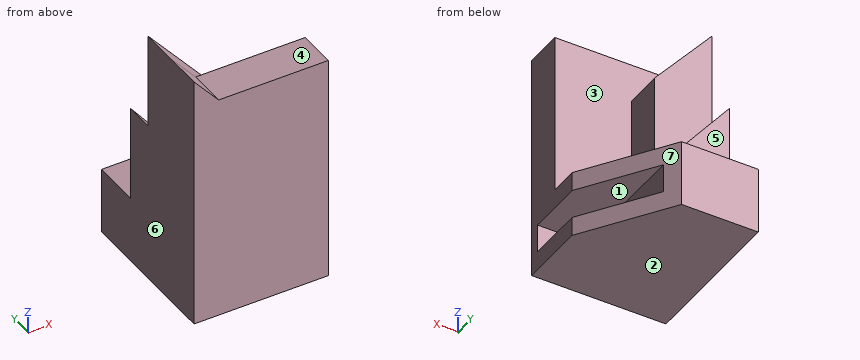
from build123d import *

# Parameters (mm, degrees)
BASE_PLATE_SKETCH_W   = 70
BASE_PLATE_SKETCH_H   = 135
BASE_PLATE_DEPTH      = 20
TOWER_DEPTH           = 35
TOWER_WINDOW_SKETCH_W = 25
TOWER_WINDOW_SKETCH_H = 15
TOWER_WINDOW_DEPTH    = 75
UPPER_STEP_DEPTH      = 35
LOWER_STEP_DEPTH      = 20
STEP_NOTCH_DEPTH      = 20


with BuildPart() as part:
    # Base Plate Sketch → Base Plate (new body)
    with BuildSketch(Plane(origin=(0, 0, 0), x_dir=(1, 0, 0), z_dir=(0, 1, 0))):
        Rectangle(BASE_PLATE_SKETCH_W, BASE_PLATE_SKETCH_H)
    extrude(amount=BASE_PLATE_DEPTH)

    # Tower Profile Sketch → Tower (add)
    with BuildSketch(Plane(origin=(0, 0, -67.5), x_dir=(-1, 0, 0), z_dir=(0, 0, -1))):
        Polygon((35, 0), (35, 80), (-5, 80), (-35, 35), (-35, 0), align=None)
    extrude(amount=-TOWER_DEPTH)

    # Tower Window Sketch → Tower Window (cut)
    with BuildSketch(Plane(origin=(0, 80, 0), x_dir=(1, 0, 0), z_dir=(0, 1, 0))):
        with Locations((22.5, 50)):
            Rectangle(TOWER_WINDOW_SKETCH_W, TOWER_WINDOW_SKETCH_H)
    extrude(amount=-TOWER_WINDOW_DEPTH, mode=Mode.SUBTRACT)

    # Upper Step Sketch → Upper Step (add)
    with BuildSketch(Plane(origin=(0, 20, 0), x_dir=(1, 0, 0), z_dir=(0, 1, 0))):
        Polygon((-35, 32.5), (5, 32.5), (-35, -17.5), align=None)
    extrude(amount=UPPER_STEP_DEPTH)

    # Lower Step Sketch → Lower Step (add)
    with BuildSketch(Plane(origin=(0, 20, 0), x_dir=(1, 0, 0), z_dir=(0, 1, 0))):
        Polygon((-35, -17.5), (-35, -67.5), (-5, -32.5), (-5, 20), align=None)
    extrude(amount=LOWER_STEP_DEPTH)

    # Step Notch Sketch → Step Notch (cut)
    with BuildSketch(Plane(origin=(0, 20, 0), x_dir=(1, 0, 0), z_dir=(0, 1, 0))):
        Polygon((35, -67.5), (35, -52.5), (-22.142857143, -52.5), (-35, -67.5), align=None)
    extrude(amount=-STEP_NOTCH_DEPTH, mode=Mode.SUBTRACT)


solid = part.part
Source: CAD feature listing. Evaluate the final solid. Frame: model axes, mm. Face numbers are marked on the shaded views. A direction names the side the tool comes from. Round coordinates to 2 decimals unless told otherwise and drop trailing zeros. Loops run counter-clockwise (first coordinate to the right, second up) from the corner with the lowest first, then second, coordinate; pieces in that order, holes last. Notation, with made-up numbers: M -9,81.5 L 18,81.5 A19 ccw 18,111.5 Z; hole C -5,89 d9. An arc over 180 degrees is marked long. Return JSON: item names as keys, results as strings. Group by question number.
1. Section query C-C on z = 11.5. Output: boundary loops of the cut face in (x, y).
2. Section query A-A on x = 19.5. Output: boundary loops of the cut face in (y, z), and give its area (3 significant figures).
3. Mould query, pull axis X, two halves, no side actions, for the marked faces 5, 6 and 7. Classes: released by +X, released by -X, zero draft, split by the parting line, or undercut.
4. Section query B-B on y = 17. Output: boundary loops of the cut face in (x, z).
5. Reachability of the marked faces 1, 2, 3 and 4 from +Z, -Z, +X, -X, +Y, -Y: full face, straight path, thin tool, end or side. Return the list, or none.
6. Material intervals for line 1 along Z through (x, y) = (26.5, 45); line 2 along Z through (x, y) = (-25, 66); line 3 along Y through (x, z) = (-29, 53), sorted ascending. Write a range as from..to.
7. Section query D-D on z = -40. Output: boundary loops of the cut face in (x, y), and give its area (4 significant figures).
8. Pin query (flat end, axial travel): pin 1 (7.5 mm diameter, centred on x = 22, y = 25.5, fed in from +Z); pin 2 (5 mm diameter, centred on x = -13.5, z = -23, fed in from +Y); pin 3 (4.5 mm diameter, centred on y = 35, z = -52.5, fed in from +X); pin 4 (12 mm diameter, centred on x = 24.5, y = 70.5, fed in from -Z). Return the tip coordinate at first contact, or that it passes through.
Checks:
{
 "1": {"outline": "M -35,0 L 35,0 L 35,20 L -5,20 L -5,40 L -30.2,40 L -30.2,55 L -35,55 Z"},
 "2": {"outline": "M 0,-67.5 L 58.25,-67.5 L 58.25,-57.5 L 5,-57.5 L 5,-42.5 L 58.25,-42.5 L 58.25,-32.5 L 20,-32.5 L 20,52.5 L 0,52.5 Z", "area": "2,940 mm²"},
 "3": {"face 5": "zero draft", "face 6": "released by -X", "face 7": "released by +X"},
 "4": {"outline": "M -35,-67.5 L 35,-67.5 L 35,-57.5 L 10,-57.5 L 10,-42.5 L 35,-42.5 L 35,52.5 L -22.14,52.5 L -35,67.5 Z"},
 "5": {"face 1": "+X, +Y", "face 2": "-Z, +X, -X, +Y, -Y", "face 3": "+Z, +X, +Y", "face 4": "+Z, +X, +Y, -Y"},
 "6": {"line 1": "z = -67.5..-57.5, -42.5..-32.5", "line 2": "z = -67.5..-32.5", "line 3": "y = 0..40"},
 "7": {"outline": "M -35,0 L 35,0 L 35,35 L 5,80 L -35,80 Z", "area": "4,925 mm²"},
 "8": {"pin 1": "stops at z = -32.5", "pin 2": "stops at y = 55", "pin 3": "stops at x = 10", "pin 4": "passes through"}
}
